from build123d import *

# Parameters (mm, degrees)
SKETCH1_W                                           = 25
SKETCH1_H                                           = 570
EXTRUDE1_DEPTH                                      = 15
CHAMFER1_SIZE                                       = 1
SKETCH_1_W                                          = 20
SKETCH_1_H                                          = 570
CUT_EXTRUDE1_DEPTH                                  = 2.5
CHAMFER2_SIZE                                       = 1
M5_TAPPED_HOLE1_D                                   = 4.2
M5_TAPPED_HOLE1_DEPTH                               = 14
M5_TAPPED_HOLE1_TIP                                 = 1.2618073
HOLE_SIZE_PER_SOCKET_HEAD_CAP_SCREW_TYP_D           = 5.5
HOLE_SIZE_PER_SOCKET_HEAD_CAP_SCREW_TYP_CBORE_D     = 10
HOLE_SIZE_PER_SOCKET_HEAD_CAP_SCREW_TYP_CBORE_DEPTH = 8
LPATTERN1_COUNT                                     = 9
LPATTERN1_PITCH                                     = 60


with BuildPart() as part:
    # Sketch1 → Extrude1 (new, symmetric)
    with BuildSketch(Plane.XY):
        Rectangle(SKETCH1_W, SKETCH1_H)
    extrude(amount=EXTRUDE1_DEPTH, both=True)

    # Chamfer1
    chamfer1_edges = [part.edges().sort_by_distance(p)[0] for p in [
        (-12.5, 285, 0),
        (12.5, 285, 0),
        (12.5, -285, 0),
        (-12.5, -285, 0),
    ]]
    chamfer(chamfer1_edges, length=CHAMFER1_SIZE)

    # 草图1 → Cut-Extrude1 (cut)
    with BuildSketch(Plane.XY.offset(15)):
        with Locations((-2.5, 0)):
            Rectangle(SKETCH_1_W, SKETCH_1_H)
    extrude(amount=-CUT_EXTRUDE1_DEPTH, mode=Mode.SUBTRACT)

    # Chamfer2
    chamfer2_edges = [part.edges().sort_by_distance(p)[0] for p in [
        (12.5, 0, -15),
        (-12.5, 0, -15),
    ]]
    chamfer(chamfer2_edges, length=CHAMFER2_SIZE)

    # M5 Tapped Hole1
    with Locations(Plane.XY.offset(12.5)):
        with Locations((-2.5, -270), (-2.5, -210), (-2.5, -150), (-2.5, -90), (-2.5, -30), (-2.5, 30), (-2.5, 90), (-2.5, 150), (-2.5, 210), (-2.5, 270)):
            Hole(M5_TAPPED_HOLE1_D / 2, depth=M5_TAPPED_HOLE1_DEPTH)
            with Locations((0, 0, -(M5_TAPPED_HOLE1_DEPTH + M5_TAPPED_HOLE1_TIP / 2))):  # 118° drill point
                Cone(0, M5_TAPPED_HOLE1_D / 2, M5_TAPPED_HOLE1_TIP, mode=Mode.SUBTRACT)

    # Hole size (per socket head cap screw type)1 (through all)
    with Locations(Plane.XY.offset(12.5)):
        with Locations((-2.5, 240)):
            hole_size_per_socket_head_cap_screw_typ = CounterBoreHole(HOLE_SIZE_PER_SOCKET_HEAD_CAP_SCREW_TYP_D / 2, HOLE_SIZE_PER_SOCKET_HEAD_CAP_SCREW_TYP_CBORE_D / 2, HOLE_SIZE_PER_SOCKET_HEAD_CAP_SCREW_TYP_CBORE_DEPTH)

    # LPattern1: Hole size (per socket head cap screw type)1 ×9
    with Locations(*[(0, -i * LPATTERN1_PITCH, 0) for i in range(1, LPATTERN1_COUNT)]):
        add(hole_size_per_socket_head_cap_screw_typ, mode=Mode.SUBTRACT)


solid = part.part
Read the model definition and answer for the solid it produces. Units are mm, in the model's axes. A direction names the side the tool comes from. Round coordinates to 2 decimals unless told otherwise and drop trailing zeros. Loops run counter-clockwise (first coordinate to the right, second up) from the corner with the lowest first, then second, coordinate; pieces in that order, holes last.
Q1. Which of the six approach directions +Z, -Z, +X, -X, +Y, -Y give full straight-line access (tool end or side, diameter ignored) to faces 1 (the face through (0, -182, 4.5)), 2 (the face through (12.5, -4, 1))?
Q2. Each of these flat-tipped pins is pushed along its axis until it touches: pin 1 (1.2 mm diameter, centred on y = 109, z = 14, fed in from -X); pin 2 (6 mm diameter, centred on x = -2.5, y = -240, fed in from +Z); pin 3 (5 mm diameter, centred on x = -4, y = 221, fed in from +Z). Where does it stop, or does it pass through?
Q3. Section A-A on y = 99 is taken. Write down the section's boundary in (x, z), and give its area (3 significant figures).
Q4. Consider probe 1 along X at (y, z) = (-240.5, -4); probe 2 along X at (y, z) = (270, 3.25); probe 3 along Z at (x, y) = (3.5, 120). Determine where each line is inside the solid, lowest interval first.
Q5. Determine the mould class of faces 3 (the face through (0, -242, 4.5)), 4 (the face through (0, -285, 0)), 5 (the face through (-12.5, -4, -1)) for opening direction X: released by +X, released by -X, zero draft, split by the parting line, or undercut.
Output:
1. face 1: +Z
1. face 2: +Z, -Z, +X, +Y, -Y
2. pin 1: stops at x = 7.5
2. pin 2: stops at z = 4.5
2. pin 3: stops at z = 12.5
3. outline: (-12.5, -14) - (-11.5, -15) - (11.5, -15) - (12.5, -14) - (12.5, 15) - (7.5, 15) - (7.5, 12.5) - (-12.5, 12.5) - close
3. area: 699 mm2
4. probe 1: x = -12.5 to -5.2, 0.2 to 12.5
4. probe 2: x = -12.5 to -4.6, -0.4 to 12.5
4. probe 3: z = -15 to 12.5
5. face 3: undercut
5. face 4: zero draft
5. face 5: released by -X
